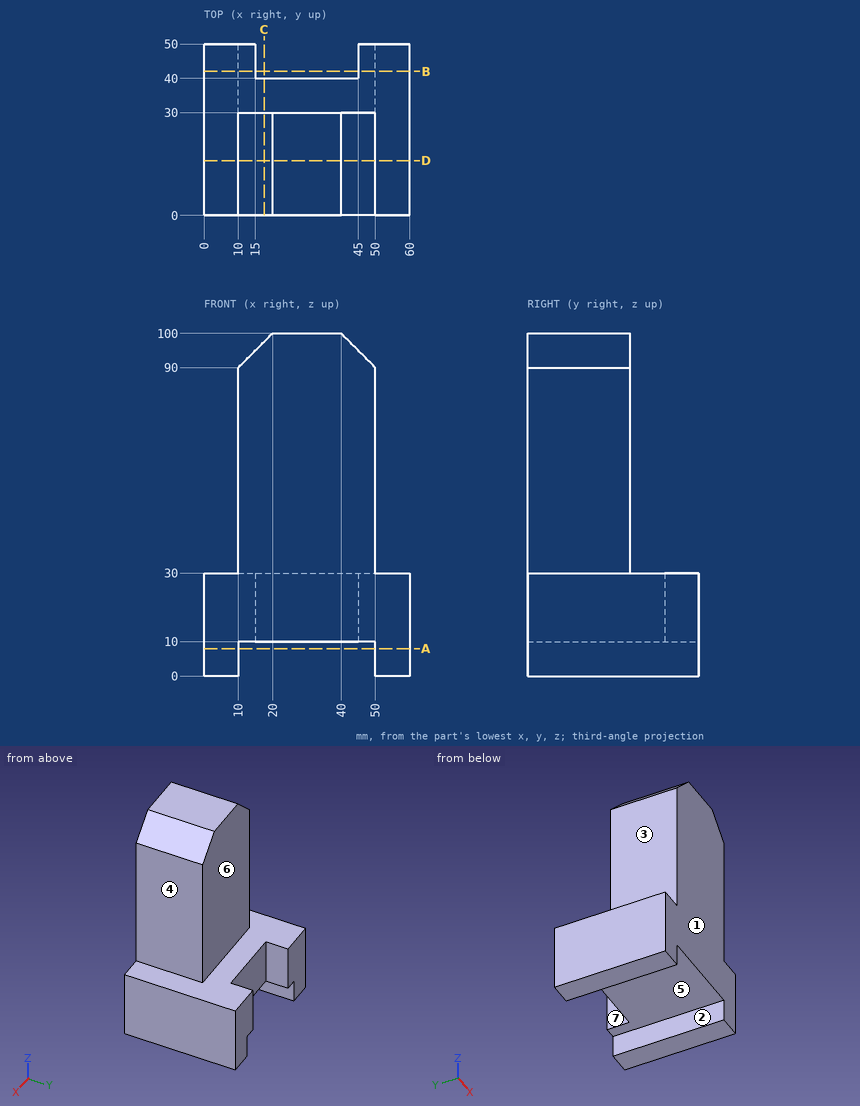
Design review of the part shown in the three views and the two pictorial views. Dimensions are in mm from the part's minimum x, y and z. A direction names the side the tool comes from. Coordinates: 2 decimals unless noted, no trailing zeros. Order: outer loops, then holes, each group sorted by start corner. A loop starts at its lowest first (then second) coordinate and runs counter-clockwise, first axis right, second up.
1) Take a section at D-D, the plane y = 16. Give the boundary of the cut face in (x, z), and give its area (3 significant figures).
2) For the marked faces 4, 5, 6 and 7, list the 3-axis set-ups (+Z, -Z, +X, -X, +Y, -Y) from which the entire face can be reached by the end or side of a thin tool; tool diameter is ignored.
3) Clearance check with flat-ended pins moving along their axes: pin 1 (8 mm diameter, centred on y = 37.5, z = 63, fed in from -X); pin 2 (12 mm diameter, centred on x = 22.5, z = 55, fed in from +Y); pin 3 (3 mm diameter, centred on x = 16.5, y = 21, fed in from -Z); pin 4 (5 mm diameter, centred on y = 30, z = 88, fed in from +X). State where each tip first meets the part, or that it passes through.
4) Take a section at C-C, the plane x = 17.5. Give the boundary of the cut face in (y, z), and give its area (4 significant figures).
5) Take a section at B-B, the plane y = 42. Give the boundary of the cut face in (x, z).
6) Wall thickness on line 1 along X through (y, z) = (14, 8.5); line 2 along Y through (x, z) = (40.5, 95.5); line 3 along Z through (x, y) = (21.5, 19): over which ranges is each line inside the solid? List them lowest first.
7) Mouldability with a two-part tool opening along X and no side actions: class the marked faces 1, 2 and 3 as +X half, -X half, draft (parallel to the pull), parting line (faces both ways), or undercut.
8) Take a section at A-A, the plane z = 8. Give the boundary of the cut face in (x, y).
Returned:
1. outline: (0, 0) - (10, 0) - (10, 10) - (50, 10) - (50, 0) - (60, 0) - (60, 30) - (50, 30) - (50, 90) - (40, 100) - (20, 100) - (10, 90) - (10, 30) - (0, 30) - close
1. area: 4,100 mm2
2. face 4: +Z, +X, +Y, -Y
2. face 5: -Z, +Y, -Y
2. face 6: +Z, +X, -X, +Y
2. face 7: +Z, -Z, +Y
3. pin 1: passes through
3. pin 2: stops at y = 30
3. pin 3: stops at z = 10
3. pin 4: stops at x = 50
4. outline: (0, 10) - (40, 10) - (40, 30) - (30, 30) - (30, 97.5) - (0, 97.5) - close
4. area: 2,825 mm2
5. outline: (0, 0) - (10, 0) - (10, 10) - (15, 10) - (15, 30) - (0, 30) - close; (45, 10) - (50, 10) - (50, 0) - (60, 0) - (60, 30) - (45, 30) - close
6. line 1: x = 0 to 10, 50 to 60
6. line 2: y = 0 to 30
6. line 3: z = 10 to 100
7. face 1: draft
7. face 2: undercut
7. face 3: -X half
8. outline: (0, 0) - (10, 0) - (10, 50) - (0, 50) - close; (50, 0) - (60, 0) - (60, 50) - (50, 50) - close
